```python
from build123d import *

# Parameters (mm, degrees)
CHAMFER1_SIZE = 1


with BuildPart() as part:
    # Sketch1 → Revolve1 (revolve)
    with BuildSketch(Plane(origin=(0, 0, 0), x_dir=(0, 0, -1), z_dir=(1, 0, 0)), mode=Mode.PRIVATE) as revolve1_sk:
        Polygon((20, 0), (20, 10), (15, 10), (15, 6.25), (0, 6.25), (0, 0), align=None)
    revolve(revolve1_sk.sketch.rotate(Axis((0, 0, 0), (0, 0, -1)), 90), axis=Axis((0, 0, 0), (0, 0, -1)))

    # Chamfer1
    chamfer1_edges = [part.edges().sort_by_distance(p)[0] for p in [
        (-6.25, 0, 0),
        (-10, 0, -15),
        (-10, 0, -20),
    ]]
    chamfer(chamfer1_edges, length=CHAMFER1_SIZE)


solid = part.part
```
Read the model definition and answer for the solid it produces. Units are mm, in the model's axes. A direction names the side the tool comes from. Coordinates: 2 decimals unless noted, no trailing zeros. Write each loop counter-clockwise with the first axis right and the second up, starting at its lowest first coordinate (ties: lowest second). Pieces come first, ordered by that corner, then holes. Notation, with made-up numbers: (16, 26) -> (34, 26) arc R21 ccw to (34, 36) -> close; hole circle Ø3 at (-34.5, -30.75). An arc over 180 degrees is marked (long way). Return JSON: item names as keys, results as strings.
1. Find the intervals of material crossed by line 1 along X through (y, z) = (-0.25, -17.75); line 2 along Z through (x, y) = (2.25, -7); line 3 along X through (y, z) = (-3.5, -18), in increasing order. Write a range as from..to.
Found:
{"line 1": "-10..10", "line 2": "-20..-15", "line 3": "-9.37..9.37"}
2. A cutting plane is placed at C-C (z = -12). Determine the outline of the cut face in (x, y).
Found:
{"outline": "circle Ø12.5 at (0, 0)"}
3. A cutting plane is placed at A-A (y = 0). Determine the outline of the cut face in (x, z).
Found:
{"outline": "(-10, -19) -> (-9, -20) -> (9, -20) -> (10, -19) -> (10, -16) -> (9, -15) -> (6.25, -15) -> (6.25, -1) -> (5.25, 0) -> (-5.25, 0) -> (-6.25, -1) -> (-6.25, -15) -> (-9, -15) -> (-10, -16) -> close"}
4. A tool of negligible diameter and unlimited length cuts with its end or side. For faces 1 (the face through (5.96, -1.88, -7.9)), 2 (the face through (0, 0, 0)), from which of +Z, -Z, +X, -X, +Y, -Y can it reach the whole face along a straight path? Write none if from no direction.
Found:
{"face 1": "+Z", "face 2": "+Z, +X, -X, +Y, -Y"}
5. Each of these flat-tipped pins is pushed along its axis until it touches: P1, Ø1, axis at x = -1, z = -7, coming from the -Y side; P2, Ø6, axis at y = -7, z = -15.5, coming from the -X side; P3, Ø1, axis at x = 3.5, z = -17.5, coming from the -Y side. Where does it stop, or does it pass through?
Found:
{"P1": "y = -6.23", "P2": "x = -9.15", "P3": "y = -9.54"}
